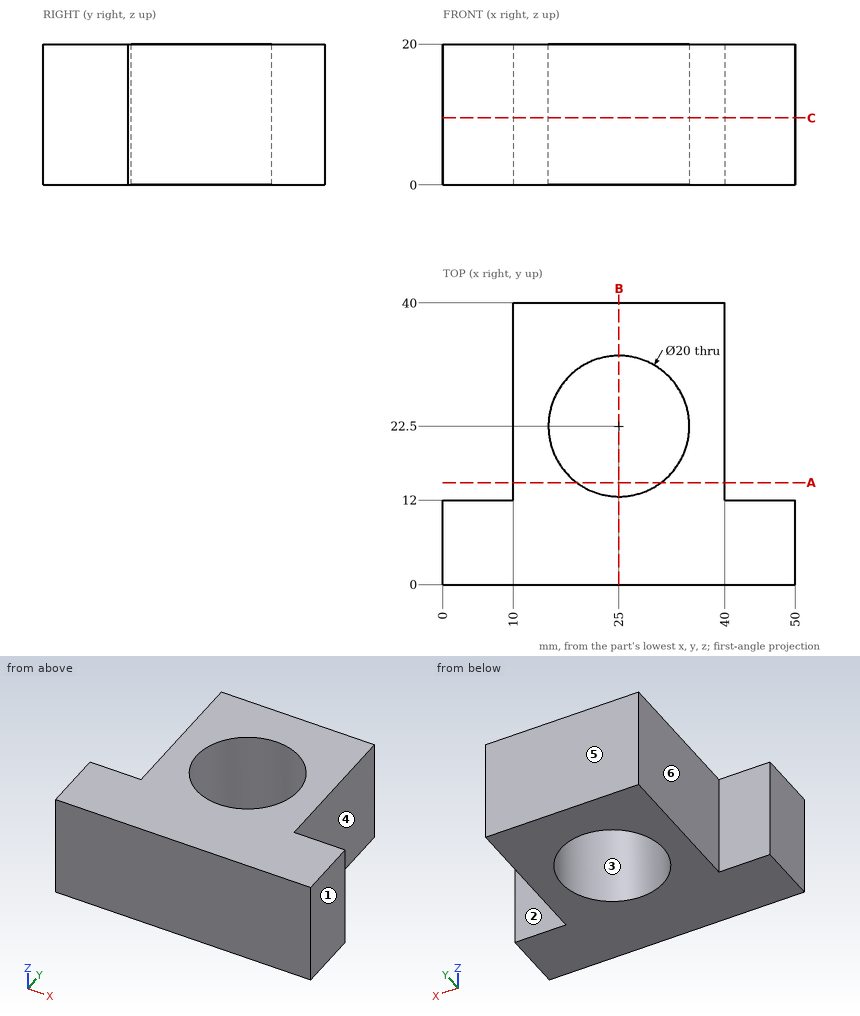
Study the drawing (mm; zero at the part's minimum x, y, z) and answer. A direction names the side the tool comes from. Round coordinates to 2 decimals unless told otherwise and drop trailing zeros. Write each loop counter-clockwise with the first axis right and the second up, starting at its lowest first coordinate (ties: lowest second). Pieces come first, ordered by that corner, then holes.
1) Flat-ended cylindrical pins translate along their axes: P1, Ø12, axis at x = 43.5, y = 7.5, coming from the -Z side; P2, Ø8, axis at x = 46, z = 8.5, coming from the +Y side; P3, Ø10, axis at y = 23, z = 7, coming from the -X side. Find the tip coordinate at first contact, or state that the pin passes through.
2) A cutting plane is placed at B-B on x = 25. Determine the outline of the cut face in (y, z), and give its area (3 significant figures).
3) Which of the six approach directions +Z, -Z, +X, -X, +Y, -Y give full straight-line access (tool end or side, diameter ignored) to the marked faces 4, 5 and 6?
4) Consider probe 1 along Y at (x, z) = (25, 8.5); probe 2 along Y at (x, z) = (32, 4.75); probe 3 along Y at (x, z) = (9.5, 14.5). Determine where each line is inside the solid, lowest interval first.
5) Determine the mould class of the marked faces 1, 2 and 3 for opening direction X: pulls with the +X half, pulls with the -X half, needs draft (parallel to the pull), parting line crosses it, or undercut.
6) A cutting plane is placed at A-A on y = 14.5. Determine the outline of the cut face in (x, z).
7) A cutting plane is placed at C-C on z = 9.5. Determine the outline of the cut face in (x, y), and give its area (3 significant figures).
Entries:
1. P1: stops at z = 0
1. P2: stops at y = 12
1. P3: stops at x = 10
2. outline: (0, 0) - (12.5, 0) - (12.5, 20) - (0, 20) - close; (32.5, 0) - (40, 0) - (40, 20) - (32.5, 20) - close
2. area: 400 mm2
3. face 4: +Z, -Z, +X, +Y
3. face 5: +Z, -Z, +X, -X, +Y
3. face 6: +Z, -Z, -X, +Y
4. probe 1: y = 0 to 12.5, 32.5 to 40
4. probe 2: y = 0 to 15.36, 29.64 to 40
4. probe 3: y = 0 to 12
5. face 1: pulls with the +X half
5. face 2: needs draft
5. face 3: undercut
6. outline: (10, 0) - (19, 0) - (19, 20) - (10, 20) - close; (31, 0) - (40, 0) - (40, 20) - (31, 20) - close
7. outline: (0, 0) - (50, 0) - (50, 12) - (40, 12) - (40, 40) - (10, 40) - (10, 12) - (0, 12) - close; hole circle Ø20 at (25, 22.5)
7. area: 1,130 mm2
